Design review of the part built by this model. Coordinates are the model's own, in mm. Face numbers are marked on the shaded views. A direction names the side the tool comes from. Round coordinates to 2 decimals unless told otherwise and drop trailing zeros. Order: outer loops, then holes, each group sorted by start corner. A loop starts at its lowest first (then second) coordinate and runs counter-clockwise, first axis right, second up. Notation, with made-up numbers: M 18,61 L 63,61 A25 cw 63,84 Z; hole C 73.5,55 d1. An arc over 180 degrees is marked long. Use a Markdown table: item, result. Add a question column.
(1) The part is to be moulded in two halves that separate along X. For the marked faces 3, 4, 5 and 6, say which applies: released by +X, released by -X, zero draft, split by the parting line, or undercut.
(2) Take a section at A-A (z = 0). Write out the cut boundary in (x, y).
(3) For pin 1 (5 mm diameter, centred on x = -0.5, y = -1, fed in from +Z); pin 2 (5 mm diameter, centred on x = 0, y = 0, fed in from -Z); pin 3 (2 mm diameter, centred on x = 20.5, y = 13, fed in from -Z), all flat-tipped, find the tip position at first contact; note any pin that passes through.
(4) Machinability: for the marked faces 1 and 2, which of the approach directions +Z, -Z, +X, -X, +Y, -Y give a long, thin tool a straight path to every point of the face, cutting with its end or side? Answer none if there is none.
(5) Take a section at C-C (x = 0). Write out the cut boundary in (y, z), then the cut area to 3 significant figures.
(6) To check wall thickness, follow probe 1 along X at (y, z) = (-1.5, 0.25); probe 2 along X at (y, z) = (13, -6); probe 3 along Y at (x, z) = (-20.5, -8.3). State the ranges of each line that lie inside material, in increasing order. Write a range as from..to.
(7) Take a section at D-D (x = 20.5). Write out the cut boundary in (y, z).
(8) Take a section at B-B (y = -8). Write out the cut boundary in (x, z).
```python
from build123d import *

# Parameters (mm, degrees)
SKETCH1_W                               = 70
SKETCH1_H                               = 35
BOSS_EXTRUDE1_DEPTH                     = 9
CUT_EXTRUDE1_DEPTH                      = 10
SKETCH3_R                               = 6
CUT_EXTRUDE2_DEPTH                      = 51.309044912
M3_TAPPED_HOLE1_REACH                   = 45.073
M3_TAPPED_HOLE1_BORE_R                  = 1.25
CBORE_FOR_M3_HEX_HEAD_BOLT1_D           = 3.5
CBORE_FOR_M3_HEX_HEAD_BOLT1_CBORE_D     = 6
CBORE_FOR_M3_HEX_HEAD_BOLT1_CBORE_DEPTH = 3
CUT_EXTRUDE3_START                      = -3
SKETCH9_R                               = 3
CUT_EXTRUDE3_DEPTH                      = 3
CHAMFER1_SIZE                           = 1
CHAMFER2_SIZE                           = 0.5


with BuildPart() as part:
    # Sketch1 → Boss-Extrude1 (new, symmetric)
    with BuildSketch(Plane.XY):
        Rectangle(SKETCH1_W, SKETCH1_H)
    extrude(amount=BOSS_EXTRUDE1_DEPTH, both=True)

    # Sketch2 → Cut-Extrude1 (cut)
    with BuildSketch(Plane.XY.offset(9)):
        with BuildLine():
            Line((-9.5, 12.5), (9.5, 12.5))
            ThreePointArc((9.5, 12.5), (11.621320344, 11.621320344), (12.5, 9.5))
            Line((12.5, 9.5), (12.5, -9.5))
            ThreePointArc((12.5, -9.5), (11.621320344, -11.621320344), (9.5, -12.5))
            Line((9.5, -12.5), (-9.5, -12.5))
            ThreePointArc((-9.5, -12.5), (-11.621320344, -11.621320344), (-12.5, -9.5))
            Line((-12.5, -9.5), (-12.5, 9.5))
            ThreePointArc((-12.5, 9.5), (-11.621320344, 11.621320344), (-9.5, 12.5))
        make_face()
    extrude(amount=-CUT_EXTRUDE1_DEPTH, mode=Mode.SUBTRACT)

    # Sketch3 → Cut-Extrude2 (cut, through all)
    with BuildSketch(Plane(origin=(0, 17.5, 0), x_dir=(1, 0, 0), z_dir=(0, 1, 0))):
        with Locations(Location((-20.5, 0, 0), (0, 0, 270))):
            Circle(SKETCH3_R)
        with Locations(Location((20.5, 0, 0), (0, 0, 270))):
            Circle(SKETCH3_R)
    extrude(amount=-CUT_EXTRUDE2_DEPTH, mode=Mode.SUBTRACT)

    # M3 Tapped Hole1 bore → M3 Tapped Hole1 (cut, up to next)
    with BuildSketch(Plane(origin=(0, 0, -9), x_dir=(-1, 0, 0), z_dir=(0, 0, -1)), mode=Mode.PRIVATE) as m3_tapped_hole1_sk1:
        with Locations((-20.5, 13)):
            Circle(M3_TAPPED_HOLE1_BORE_R)
    m3_tapped_hole1_tool1 = extrude(m3_tapped_hole1_sk1.sketch, amount=-M3_TAPPED_HOLE1_REACH, mode=Mode.PRIVATE) & part.part
    # M3 Tapped Hole1 bore → M3 Tapped Hole1 (cut, up to next)
    with BuildSketch(Plane(origin=(0, 0, -9), x_dir=(-1, 0, 0), z_dir=(0, 0, -1)), mode=Mode.PRIVATE) as m3_tapped_hole1_sk2:
        with Locations((-20.5, -13)):
            Circle(M3_TAPPED_HOLE1_BORE_R)
    m3_tapped_hole1_tool2 = extrude(m3_tapped_hole1_sk2.sketch, amount=-M3_TAPPED_HOLE1_REACH, mode=Mode.PRIVATE) & part.part
    # M3 Tapped Hole1 bore → M3 Tapped Hole1 (cut, up to next)
    with BuildSketch(Plane(origin=(0, 0, -9), x_dir=(-1, 0, 0), z_dir=(0, 0, -1)), mode=Mode.PRIVATE) as m3_tapped_hole1_sk3:
        with Locations((20.5, -13)):
            Circle(M3_TAPPED_HOLE1_BORE_R)
    m3_tapped_hole1_tool3 = extrude(m3_tapped_hole1_sk3.sketch, amount=-M3_TAPPED_HOLE1_REACH, mode=Mode.PRIVATE) & part.part
    # M3 Tapped Hole1 bore → M3 Tapped Hole1 (cut, up to next)
    with BuildSketch(Plane(origin=(0, 0, -9), x_dir=(-1, 0, 0), z_dir=(0, 0, -1)), mode=Mode.PRIVATE) as m3_tapped_hole1_sk4:
        with Locations((20.5, 13)):
            Circle(M3_TAPPED_HOLE1_BORE_R)
    m3_tapped_hole1_tool4 = extrude(m3_tapped_hole1_sk4.sketch, amount=-M3_TAPPED_HOLE1_REACH, mode=Mode.PRIVATE) & part.part
    add(m3_tapped_hole1_tool1.solids().sort_by_distance((20.5, 13, -9))[0], mode=Mode.SUBTRACT)
    add(m3_tapped_hole1_tool2.solids().sort_by_distance((20.5, -13, -9))[0], mode=Mode.SUBTRACT)
    add(m3_tapped_hole1_tool3.solids().sort_by_distance((-20.5, -13, -9))[0], mode=Mode.SUBTRACT)
    add(m3_tapped_hole1_tool4.solids().sort_by_distance((-20.5, 13, -9))[0], mode=Mode.SUBTRACT)

    # CBORE for M3 Hex Head Bolt1 (through all)
    with Locations(Plane(origin=(-21.223251094, -7.58728159, -1), x_dir=(1, 0, 0), z_dir=(0, 0, 1))):
        with Locations((21.223251094, 7.58728159)):
            CounterBoreHole(CBORE_FOR_M3_HEX_HEAD_BOLT1_D / 2, CBORE_FOR_M3_HEX_HEAD_BOLT1_CBORE_D / 2, CBORE_FOR_M3_HEX_HEAD_BOLT1_CBORE_DEPTH)

    # Sketch9 → Cut-Extrude3 (cut)
    with BuildSketch(Plane(origin=(0, 0, -9), x_dir=(-1, 0, 0), z_dir=(0, 0, -1)).offset(CUT_EXTRUDE3_START)):
        with Locations(Location((0, 0, 0), (0, 0, 180))):
            Circle(SKETCH9_R)
    extrude(amount=CUT_EXTRUDE3_DEPTH, mode=Mode.SUBTRACT)

    # Chamfer1
    chamfer1_edges = [part.edges().sort_by_distance(p)[0] for p in [
        (-35, 0, 9),
        (35, 0, 9),
        (-35, 0, -9),
        (35, 0, -9),
    ]]
    chamfer(chamfer1_edges, length=CHAMFER1_SIZE)

    # Chamfer2
    chamfer2_edges = [part.edges().sort_by_distance(p)[0] for p in [
        (-20.5, -17.5, -6),
        (-20.5, 17.5, -6),
        (20.5, -17.5, -6),
        (20.5, 17.5, -6),
    ]]
    chamfer(chamfer2_edges, length=CHAMFER2_SIZE)


solid = part.part
```
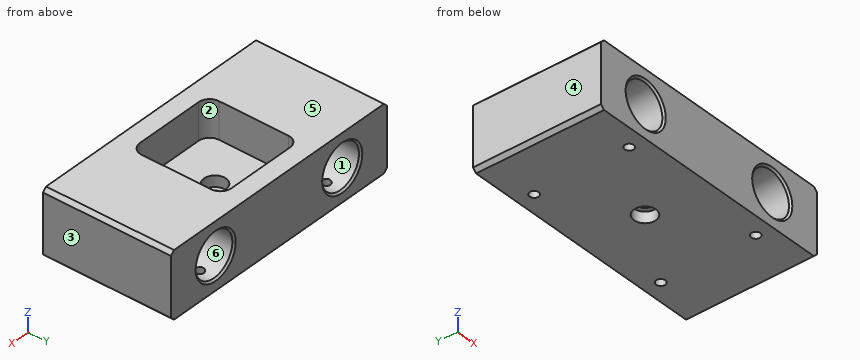
Verdict:
| question | item | result |
|---|---|---|
| 1 | face 3 | released by +X |
| 1 | face 4 | released by -X |
| 1 | face 5 | zero draft |
| 1 | face 6 | undercut |
| 2 | outline | M -35,-17.5 L -27,-17.5 L -26.5,-17 L -26.5,17 L -27,17.5 L -35,17.5 Z; M -14.5,-17 L -14,-17.5 L 14,-17.5 L 14.5,-17 L 14.5,17 L 14,17.5 L -14,17.5 L -14.5,17 Z; M 26.5,-17 L 27,-17.5 L 35,-17.5 L 35,17.5 L 27,17.5 L 26.5,17 Z; hole M -12.5,-9.5 A3 ccw -9.5,-12.5 L 9.5,-12.5 A3 ccw 12.5,-9.5 L 12.5,9.5 A3 ccw 9.5,12.5 L -9.5,12.5 A3 ccw -12.5,9.5 Z |
| 3 | pin 1 | stops at z = -1 |
| 3 | pin 2 | stops at z = -6 |
| 3 | pin 3 | stops at z = 5.92 |
| 4 | face 1 | +Y, -Y |
| 4 | face 2 | +Z |
| 5 | outline | M -17.5,-9 L -3,-9 L -3,-6 L -1.75,-6 L -1.75,-4 L -3,-4 L -3,-1 L -12.5,-1 L -12.5,9 L -17.5,9 Z; M 1.75,-6 L 3,-6 L 3,-9 L 17.5,-9 L 17.5,9 L 12.5,9 L 12.5,-1 L 3,-1 L 3,-4 L 1.75,-4 Z |
| 5 | area | 337 mm^2 |
| 6 | probe 1 | x = -35..-26.49, -14.51..-12.5, 12.5..14.51, 26.49..35 |
| 6 | probe 2 | x = -35..-21.75, -19.25..19.25, 21.75..35 |
| 6 | probe 3 | y = -17.5..-14.25, -11.75..11.75, 14.25..17.5 |
| 7 | outline | M -17.5,-9 L -14.25,-9 L -14.25,-6 L -17,-6 L -17.5,-6.5 Z; M -17.5,6.5 L -17,6 L 17,6 L 17.5,6.5 L 17.5,9 L -17.5,9 Z; M -11.75,-9 L 11.75,-9 L 11.75,-6 L -11.75,-6 Z; M 14.25,-9 L 17.5,-9 L 17.5,-6.5 L 17,-6 L 14.25,-6 Z |
| 8 | outline | M -35,-8 L -34,-9 L 34,-9 L 35,-8 L 35,8 L 34,9 L 12.5,9 L 12.5,-1 L -12.5,-1 L -12.5,9 L -34,9 L -35,8 Z; hole C -20.5,0 d12; hole C 20.5,0 d12 |
